```python
from build123d import *

# Parameters (mm, degrees)
SKETCH1_R           = 5
SKETCH1_R_2         = 3
BOSS_EXTRUDE1_DEPTH = 4


with BuildPart() as part:
    # Sketch1 → Boss-Extrude1 (new body)
    with BuildSketch(Plane.XY):
        with BuildLine():
            Line((-6, -60), (-6, -8.660254038))
            ThreePointArc((-6, -8.660254038), (-6.275444087, -7.023619861), (-7.071428571, -5.567306167))
            ThreePointArc((-7.071428571, -5.567306167), (0, 9), (7.071428571, -5.567306167))
            ThreePointArc((7.071428571, -5.567306167), (6.275444087, -7.023619861), (6, -8.660254038))
            Line((6, -8.660254038), (6, -60))
            ThreePointArc((6, -60), (0, -66), (-6, -60))
        make_face()
        Circle(SKETCH1_R, mode=Mode.SUBTRACT)
        with Locations((0, -20)):
            Circle(SKETCH1_R_2, mode=Mode.SUBTRACT)
        with Locations((0, -60)):
            Circle(SKETCH1_R_2, mode=Mode.SUBTRACT)
    extrude(amount=BOSS_EXTRUDE1_DEPTH)


solid = part.part
```
Part model, mm, in its own coordinate system. A direction names the side the tool comes from. Round coordinates to 2 decimals unless told otherwise and drop trailing zeros. Write each loop counter-clockwise with the first axis right and the second up, starting at its lowest first coordinate (ties: lowest second). Pieces come first, ordered by that corner, then holes.
Item 1: Cut at C-C, the plane z = 1.45. Give the cut face in (x, y).
Results:
outline: (-7.07, -5.57) arc R5 cw to (-6, -8.66) - (-6, -60) arc R6 ccw to (6, -60) - (6, -8.66) arc R5 cw to (7.07, -5.57) arc R9 ccw (long way) to start; hole circle Ø10 at (0, 0); hole circle Ø6 at (0, -60); hole circle Ø6 at (0, -20)
Item 2: Probe L1, parallel to Y at x = 0, z = 2.65; L2, parallel to Y at x = -1.75, z = 3.6; L3, parallel to X at y = -31.5, z = 2.1. List the from-to ranges inside material, lowest first.
Results:
L1: y = -66 to -63, -57 to -23, -17 to -5, 5 to 9
L2: y = -65.74 to -62.44, -57.56 to -22.44, -17.56 to -4.68, 4.68 to 8.83
L3: x = -6 to 6
Item 3: Drop a flat-ended pin along its axis: pin 1 Ø2 at (y, z) = (-38.5, 2) entering from +X. Give the stop position or say it passes through.
Results:
pin 1: stops at x = 6
Item 4: Cut at B-B, the plane x = 0. Give the cut face in (y, z), plus the area to 3 significant figures.
Results:
outline: (-66, 0) - (-63, 0) - (-63, 4) - (-66, 4) - close; (-57, 0) - (-23, 0) - (-23, 4) - (-57, 4) - close; (-17, 0) - (-5, 0) - (-5, 4) - (-17, 4) - close; (5, 0) - (9, 0) - (9, 4) - (5, 4) - close
area: 212 mm2
Item 5: Two-plate mould, pull along X, no slides. Class faces 3 (the cylindrical face through (-0.65, -22.93, 1.97)), 4 (the cylindrical face through (0, -57, 2)), 5 (the flat face through (6, -34, 2)), 6 (the cylindrical face through (0, -66, 2)): +X half, -X half, draft (parallel to the pull), parting line (faces both ways), or undercut.
Results:
face 3: undercut
face 4: undercut
face 5: +X half
face 6: parting line
Item 6: Which spindle directions (+Z, -Z, +X, -X, +Y, -Y) get a long thin tool onto all of the face, cutting with end or side? Do faces 1 (the flat face through (-6, -35, 2)), 2 (the flat face through (0, -28, 4)). Say none if no direction does.
Results:
face 1: +Z, -Z, -X, -Y
face 2: +Z, +X, -X, +Y, -Y
Item 7: Cut at D-D, the plane y = -18. Give the cut face in (x, z).
Results:
outline: (-6, 0) - (-2.24, 0) - (-2.24, 4) - (-6, 4) - close; (2.24, 0) - (6, 0) - (6, 4) - (2.24, 4) - close
Item 8: Cut at A-A, the plane y = 0. Give the cut face in (x, z).
Results:
outline: (-9, 0) - (-5, 0) - (-5, 4) - (-9, 4) - close; (5, 0) - (9, 0) - (9, 4) - (5, 4) - close
